Geometry: final body of the model. Coordinates: model frame, mm. Face numbers are marked on the shaded views. Give positions to 0.01 mm unless a question says otherwise; leave off trailing zeros. Write each loop counter-clockwise with the first axis right and the second up, starting at its lowest first coordinate (ties: lowest second). Pieces come first, ordered by that corner, then holes. Notation, with made-up numbers: M -18,19 L 18,19 A20 ccw 18,44 Z; hole C 25,17 d9. An arc over 180 degrees is marked long. Answer as a JSON object with one key per item and string values.
from build123d import *

# Parameters (mm, degrees)
SKETCH_2_W            = 39.483354071
SKETCH_2_H            = 80
EXTRUDE_1_DEPTH       = 6
SKETCH_3_R            = 3
CUT_EXTRUDE_1_DEPTH   = 10
HOLE_WIZARD_1_0_1_1_D = 6.5
SKETCH_6_R            = 6.5
CUT_EXTRUDE_2_DEPTH   = 218.242322412
HOLE_WIZARD_1_0_1_2_D = 3.5


with BuildPart() as part:
    # 草图2 → 凸台-拉伸1 (new body)
    with BuildSketch(Plane(origin=(0.031845394, 0, -9.289854674), x_dir=(0.9999941245437004, 0, 0.0034279553787324732), z_dir=(-0.0034279553787324732, 0, 0.9999941245437004))):
        with Locations((-185.77882216, 30.129161482)):
            Rectangle(SKETCH_2_W, SKETCH_2_H)
    extrude(amount=EXTRUDE_1_DEPTH)

    # 草图3 → 切除-拉伸1 (cut)
    with BuildSketch(Plane(origin=(0.011277662, 0, -3.289889926), x_dir=(0.9999941245437003, 0, 0.003427955378732479), z_dir=(-0.003427955378732479, 0, 0.9999941245437004))):
        with Locations((-200.520499196, -4.870838518)):
            Circle(SKETCH_3_R)
        with Locations((-171.037145125, -4.870838518)):
            Circle(SKETCH_3_R)
    extrude(amount=-CUT_EXTRUDE_1_DEPTH, mode=Mode.SUBTRACT)

    # Ø1.0 (1) 直径孔1 (through all)
    with Locations(Plane(origin=(0.011277662, 0, -3.289889926), x_dir=(0.9999941245437003, 0, 0.003427955378732479), z_dir=(-0.003427955378732479, 0, 0.9999941245437004))):
        with Locations((-190.520499196, -4.870838518), (-181.037145125, -4.870838518)):
            Hole(HOLE_WIZARD_1_0_1_1_D / 2)

    # 草图6 → 切除-拉伸2 (cut, through all)
    with BuildSketch(Plane(origin=(0.031845394, 0, -9.289854674), x_dir=(-0.9999941245437003, 0, -0.003427955378732479), z_dir=(0.003427955378732479, 0, -0.9999941245437004))):
        with Locations((185.777574302, 51.129161482)):
            Circle(SKETCH_6_R)
    extrude(amount=-CUT_EXTRUDE_2_DEPTH, mode=Mode.SUBTRACT)

    # Ø1.0 (1) 直径孔2 (through all)
    with Locations(Plane(origin=(0.011277662, 0, -3.289889926), x_dir=(0.9999941245437003, 0, 0.003427955378732479), z_dir=(-0.003427955378732479, 0, 0.9999941245437004))):
        with Locations((-185.777574302, 65.629161482), (-171.277574302, 51.129161482), (-185.777574302, 36.629161482), (-200.277574302, 51.129161482)):
            Hole(HOLE_WIZARD_1_0_1_2_D / 2)


solid = part.part
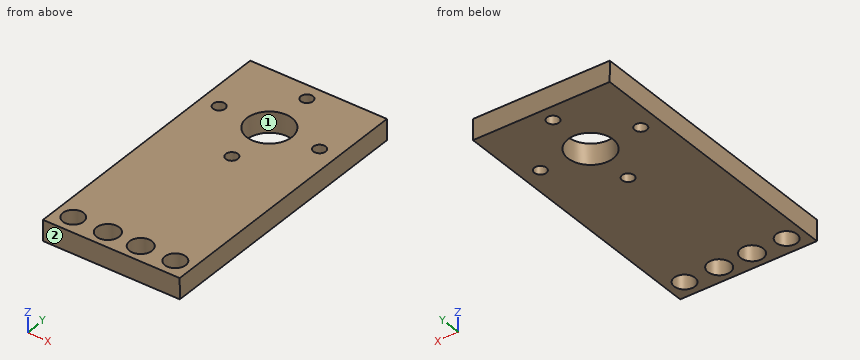
1) Cut plane B-B on y = 17.5. Return loops of the section in (x, z).
Geometry check:
{"outline": "M -205.51,-3.99 L -205.49,-9.99 L -166,-9.86 L -166.02,-3.86 Z"}
2) Pull-direction query (X, two-part tool) for the marked faces 1 and 2; classes: pulls with the +X half, pulls with the -X half, needs draft (parallel to the pull), parting line crosses it, or undercut.
Geometry check:
{"face 1": "undercut", "face 2": "needs draft"}
3) Line query: line 1 (Y direction, x = -186, z = -6.75); line 2 (Y direction, x = -190, z = -8); line 3 (Y direction, x = -200, z = -7.5). Output: solid intervals per line, ascending. Write a range as from..to.
Geometry check:
{"line 1": "y = -9.87..34.9, 38.36..44.63, 57.62..63.9, 67.36..70.13", "line 2": "y = -9.87..-8.08, -1.66..46.21, 56.05..70.13", "line 3": "y = -9.87..-7.83, -1.91..49.4, 52.86..70.13"}
4) Contact query for flat-ended pins moving along their axis: P1, Ø10, axis at x = -171, y = 20.5, coming from the -Z side; P2, Ø5, axis at x = -181.5, y = 48.5, coming from the +Z side; P3, Ø1, axis at y = 36, z = -5.5, coming from the +X side. Output: stop coordinate, or through.
Geometry check:
{"P1": "stops at z = -9.89", "P2": "stops at z = -3.9", "P3": "stops at x = -166.02"}
5) Cut plane A-A on x = -186.5. Give the number of separate pieces and of enclosed holes in the cut face, and give its area (3 significant figures).
Geometry check:
{"separate pieces": "4", "enclosed holes": "0", "area": "365 mm2"}
